Work out the finished part from the listing and answer in its coordinate system (mm). Round coordinates to 2 decimals unless told otherwise and drop trailing zeros. Order: outer loops, then holes, each group sorted by start corner. A loop starts at its lowest first (then second) coordinate and runs counter-clockwise, first axis right, second up. Notation, with made-up numbers: (53.25, -15.75) - (86.25, -15.75) arc R21 ccw to (86.25, 21.25) - close; hole circle Ø10 at (-23, -17). An arc over 180 degrees is marked (long way). Answer in a Markdown table with one row per item.
from build123d import *

# Parameters (mm, degrees)
COTTER_BODY_DEPTH = 6


with BuildPart() as part:
    # Cotter Profile Sketch → Cotter Body (new, symmetric)
    with BuildSketch(Plane.XY):
        with BuildLine():
            Line((-7.388671752, 77.068898934), (7.388671752, 77.068898934))
            ThreePointArc((7.388671752, 77.068898934), (10.962916131, 75.565293809), (12.387459643, 71.958809784))
            Line((12.387459643, 71.958809784), (9.612540357, -54.041190216))
            ThreePointArc((9.612540357, -54.041190216), (8.110147341, -57.505345445), (4.613752466, -58.931101066))
            Line((4.613752466, -58.931101066), (-4.613752466, -58.931101066))
            ThreePointArc((-4.613752466, -58.931101066), (-8.110147341, -57.505345445), (-9.612540357, -54.041190216))
            Line((-9.612540357, -54.041190216), (-12.387459643, 71.958809784))
            ThreePointArc((-12.387459643, 71.958809784), (-10.962916131, 75.565293809), (-7.388671752, 77.068898934))
        make_face()
    extrude(amount=COTTER_BODY_DEPTH, both=True)


solid = part.part
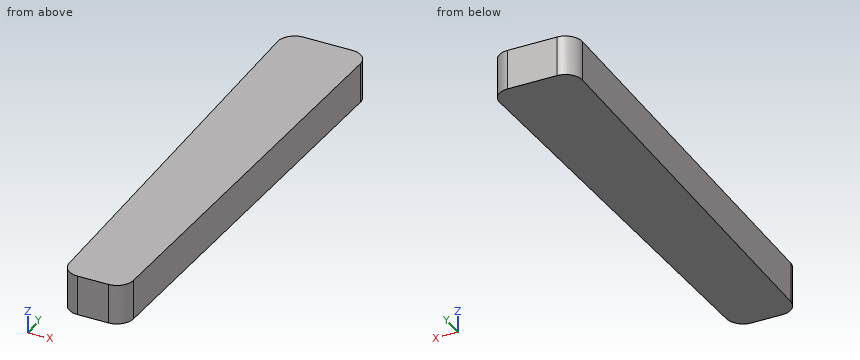
1) Find section C-C, the plane y = -48. Give the vertices of the cut face in (x, z), then the cut area to 3 significant figures.
Filled in:
| item | result |
|---|---|
| outline | (-9.75, -6) - (9.75, -6) - (9.75, 6) - (-9.75, 6) - close |
| area | 234 mm^2 |
2) Find the intervals of material crossed by probe 1 along X at (y, z) = (-34, 0); probe 2 along X at (y, z) = (63, 1.75); probe 3 along Y at (x, z) = (5, 2), in increasing order. Write a range as from..to.
Filled in:
| item | result |
|---|---|
| probe 1 | x = -10.05..10.05 |
| probe 2 | x = -12.19..12.19 |
| probe 3 | y = -58.92..77.07 |
3) Each of these flat-tipped pins is pushed along its axis until it touches: pin 1 (1 mm diameter, centred on y = -29, z = -0.5, fed in from -X); pin 2 (2 mm diameter, centred on y = 29.5, z = -1, fed in from +X); pin 3 (6 mm diameter, centred on x = 9.5, z = -1, fed in from -Y). Where does it stop, or does it pass through?
Filled in:
| item | result |
|---|---|
| pin 1 | stops at x = -10.18 |
| pin 2 | stops at x = 11.47 |
| pin 3 | stops at y = -58.56 |
4) Find section B-B, the plane y = 9.5. Give the vertices of the cut face in (x, z), then the cut area to 3 significant figures.
Filled in:
| item | result |
|---|---|
| outline | (-11.01, -6) - (11.01, -6) - (11.01, 6) - (-11.01, 6) - close |
| area | 264 mm^2 |
5) Find section A-A, the plane z = 4. Give the vertices of the cut face in (x, y), then the cut area to 3 significant figures.
Filled in:
| item | result |
|---|---|
| outline | (-12.39, 71.96) - (-9.61, -54.04) arc R5 ccw to (-4.61, -58.93) - (4.61, -58.93) arc R5 ccw to (9.61, -54.04) - (12.39, 71.96) arc R5 ccw to (7.39, 77.07) - (-7.39, 77.07) arc R5 ccw to start |
| area | 2,970 mm^2 |
